from build123d import *

# Parameters (mm, degrees)
FILLET1_R     = 2
CHAMFER1_SIZE = 0.5


with BuildPart() as part:
    # Sketch1 → Revolve1 (revolve)
    with BuildSketch(Plane.XY):
        Polygon((0, 0), (0, 4), (8, 4), (8, 3.25), (10, 3.25), (10, 4.5), (28, 4.5), (34, 6), (62, 6), (62, 0), align=None)
    revolve(axis=Axis((62, 0, 0), (-1, 0, 0)))

    # Fillet1
    fillet1_edges = [part.edges().sort_by_distance(p)[0] for p in [
        (62, -6, 0),
    ]]
    fillet(fillet1_edges, radius=FILLET1_R)

    # Chamfer1
    chamfer1_edges = [part.edges().sort_by_distance(p)[0] for p in [
        (0, -4, 0),
    ]]
    chamfer(chamfer1_edges, length=CHAMFER1_SIZE)


solid = part.part
Could you check a few things on this model? Use its own coordinates, in mm. A direction names the side the tool comes from. Round coordinates to 2 decimals unless told otherwise and drop trailing zeros. Loops run counter-clockwise (first coordinate to the right, second up) from the corner with the lowest first, then second, coordinate; pieces in that order, holes last. Notation, with made-up numbers: (-21, 18.5) - (3, 18.5) arc R23 cw to (3, 41.5) - close; hole circle Ø7 at (-19.75, -25.75). An arc over 180 degrees is marked (long way). Write item = value, one per line.
1) I need wall thicknesses on line 1 along X through (y, z) = (2, 3.25); line 2 along Y through (x, z) = (39, 0.25); line 3 along X through (y, z) = (3.75, -1.25). Which ranges of each line are inside material? Lowest first, please. Write a range as from..to.
Computed:
line_1 = 0.32..8, 10..62
line_2 = -5.99..5.99
line_3 = 0.45..8, 10..62
2) Imagine slicing it at A-A (y = 0). Please give me the cut outline in (x, z), and give its area (3 significant figures).
Computed:
outline = (0, -3.5) - (0.5, -4) - (8, -4) - (8, -3.25) - (10, -3.25) - (10, -4.5) - (28, -4.5) - (34, -6) - (60, -6) arc R2 ccw to (62, -4) - (62, 4) arc R2 ccw to (60, 6) - (34, 6) - (28, 4.5) - (10, 4.5) - (10, 3.25) - (8, 3.25) - (8, 4) - (0.5, 4) - (0, 3.5) - close
area = 636 mm2
3) If we mould it in two halves opening along X, with no side actions, what happens to faces 1 (the flat face through (8, -2, -3)), 2 (the cylindrical face through (19.13, -0.59, -4.46)), 3 (the flat face through (0, 0, 0))? For each: pulls with the +X half, pulls with the -X half, needs draft (parallel to the pull), parting line crosses it, or undercut.
Computed:
face_1 = undercut
face_2 = needs draft
face_3 = pulls with the -X half
4) I'm going to push flat-ended pins straight in: P1, Ø3, axis at x = 34, z = 2.5, coming from the -Y side; P2, Ø1.5, axis at x = 29.5, z = -4.5, coming from the -Y side; P3, Ø3, axis at x = 18, y = 2, coming from the -Z side. Where does each tip first touch, or does it pass through?
Computed:
P1 = -5.92
P2 = -3.16
P3 = -4.47
5) Imagine slicing it at C-C (x = 49.5). Please give me the cut outline in (y, z).
Computed:
outline = circle Ø12 at (0, 0)
6) On a 3-axis mill with a long thin cutter (end or side, diameter ignored), from which of +Z, -Z, +X, -X, +Y, -Y can I reach the whole of each face in a straight line? I mean faces 4 (the cylindrical face through (9.014, -2.579, 1.978)), 5 (the cylindrical face through (47, -6, 0)), 6 (the cylindrical face through (4.302, -0.867, 3.905)). Say none if no direction works.
Computed:
face_4 = none
face_5 = +X, -X
face_6 = -X
